Design review of the part built by this model. Coordinates are the model's own, in mm. Face numbers are marked on the shaded views. A direction names the side the tool comes from. Give positions to 0.01 mm unless a question says otherwise; leave off trailing zeros. Write each loop counter-clockwise with the first axis right and the second up, starting at its lowest first coordinate (ties: lowest second). Pieces come first, ordered by that corner, then holes. Notation, with made-up numbers: (19, 47) -> (58, 47) arc R29 cw to (58, 70) -> close; hole circle Ø10 at (82.5, 29). An arc over 180 degrees is marked (long way). Write each question's results on one line, items separated by ' | '. Start each with the question number.
(1) For the marked faces 1 and 2, list the 3-axis set-ups (+Z, -Z, +X, -X, +Y, -Y) from which the entire face can be reached by the end or side of a thin tool; tool diameter is ignored.
(2) Clearance check with flat-ended pins moving along their axes: pin 1 (12 mm diameter, centred on x = -2, y = 15.5, fed in from -Z); pin 2 (5 mm diameter, centred on y = 2, z = -49.5, fed in from +X); pin 3 (5 mm diameter, centred on x = -9.5, z = -48.26, fed in from +Y); pin 4 (3 mm diameter, centred on y = 1.5, z = -42, fed in from -X). State where each tip first meets the part, or that it passes through.
(3) Take a section at A-A (x = -9.5). State the section outline as (y, z) points, plus the area to 3 significant figures.
(4) Take a section at D-D (x = 0). State the section outline as (y, z) points.
(5) To check wall thickness, follow probe 1 along Z at (x, y) = (-9.5, 5.25); probe 2 along Z at (x, y) = (6, 17). State the ranges of each line that lie inside material, in increasing order.
(6) Take a section at C-C (z = -47). State the section outline as (x, y) points, plus the area to 3 significant figures.
(7) Take a section at B-B (y = 3.5). State the section outline as (x, z) points.
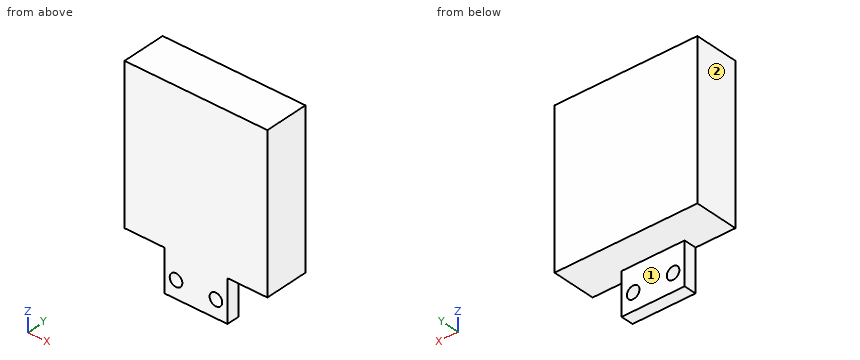
from build123d import *

# Parameters (mm, degrees)
SKETCH1_W           = 68
SKETCH1_H           = 73
BOSS_EXTRUDE1_DEPTH = 21
SKETCH2_W           = 30
SKETCH2_H           = 6.020166846
BOSS_EXTRUDE2_DEPTH = 20
SKETCH3_R           = 3
CUT_EXTRUDE1_DEPTH  = 20


with BuildPart() as part:
    # Sketch1 → Boss-Extrude1 (new body)
    with BuildSketch(Plane(origin=(0, 0, 0), x_dir=(1, 0, 0), z_dir=(0, 1, 0))):
        Rectangle(SKETCH1_W, SKETCH1_H)
    extrude(amount=BOSS_EXTRUDE1_DEPTH)

    # Sketch2 → Boss-Extrude2 (add)
    with BuildSketch(Plane(origin=(0, 0, -36.5), x_dir=(-1, 0, 0), z_dir=(0, 0, -1))):
        with Locations((0, 3.010083423)):
            Rectangle(SKETCH2_W, SKETCH2_H)
    extrude(amount=BOSS_EXTRUDE2_DEPTH)

    # Sketch3 → Cut-Extrude1 (cut)
    with BuildSketch(Plane(origin=(0, 6.020166846, 0), x_dir=(1, 0, 0), z_dir=(0, 1, 0))):
        with Locations(Location((9.5, 48.256848867, 0), (0, 0, 180))):
            Circle(SKETCH3_R)
        with Locations(Location((-9.5, 48.256848867, 0), (0, 0, 180))):
            Circle(SKETCH3_R)
    extrude(amount=-CUT_EXTRUDE1_DEPTH, mode=Mode.SUBTRACT)


solid = part.part
Report:
1) face 1: -Z, +X, -X, +Y | face 2: +Z, -Z, -X, +Y, -Y
2) pin 1: z = -36.5 | pin 2: x = 15 | pin 3: through | pin 4: x = -15
3) outline: (0, -56.5) -> (6.02, -56.5) -> (6.02, -51.26) -> (0, -51.26) -> close; (0, -45.26) -> (6.02, -45.26) -> (6.02, -36.5) -> (21, -36.5) -> (21, 36.5) -> (0, 36.5) -> close | area: 1,620 mm2
4) outline: (0, -56.5) -> (6.02, -56.5) -> (6.02, -36.5) -> (21, -36.5) -> (21, 36.5) -> (0, 36.5) -> close
5) probe 1: -56.5 to -51.26, -45.26 to 36.5 | probe 2: -36.5 to 36.5
6) outline: (-15, 0) -> (-12.22, 0) -> (-12.22, 6.02) -> (-15, 6.02) -> close; (-6.78, 0) -> (6.78, 0) -> (6.78, 6.02) -> (-6.78, 6.02) -> close; (12.22, 0) -> (15, 0) -> (15, 6.02) -> (12.22, 6.02) -> close | area: 115 mm2
7) outline: (-34, -36.5) -> (-15, -36.5) -> (-15, -56.5) -> (15, -56.5) -> (15, -36.5) -> (34, -36.5) -> (34, 36.5) -> (-34, 36.5) -> close; hole circle Ø6 at (-9.5, -48.26); hole circle Ø6 at (9.5, -48.26)
